Verification items for the finished model (mm, model axes). A direction names the side the tool comes from. Coordinates: 2 decimals unless noted, no trailing zeros. Order: outer loops, then holes, each group sorted by start corner. A loop starts at its lowest first (then second) coordinate and runs counter-clockwise, first axis right, second up. Notation, with made-up numbers: M 59.25,-2.75 L 89.25,-2.75 A34 ccw 89.25,28.25 Z; hole C -27,2.25 d5. An arc over 180 degrees is marked long. Return JSON: item names as keys, results as strings. Group by question number.
Q1. Access from +Z, -Z, +X, -X, +Y, -Y to the whole of each face (thin tool, end or side, straight path). Record for faces 1 (the face through (5.3, 0.2, 0)), 2 (the face through (11.215, 11.199, -3.042)).
Q2. Section check A-A, the plane y = 0. Enter the section's corners in (x, z), then the cut area to 3 significant figures.
Q3. Section check D-D, the plane y = 9. Enter the section's corners in (x, z), then the cut area to 3 significant figures.
Q4. Thickness scan on probe 1 along Z at (x, y) = (-0.75, -8.5); probe 2 along Y at (x, z) = (4, 14.5); probe 3 along Y at (x, z) = (4.5, 7). Record the ranges inside material, lowest first.
Q5. Section check C-C, the plane z = 21.5. Enter the section's corners in (x, y), then the cut area to 3 significant figures.
Q6. Go/stop test with flat-tipped pins: pin 1 Ø6 at (y, z) = (-6, 4.5) entering from +X; pin 2 Ø2 at (x, z) = (3, 15) entering from +Y; pin 3 Ø3 at (y, z) = (6, 10.5) entering from -X; pin 4 Ø11.5 at (x, y) = (-5.5, 3) entering from +Z. Record where each tip stops, or that it passes through.
from build123d import *

# Parameters (mm, degrees)
SKETCH_1_R      = 5
EXTRUDE_1_DEPTH = 25
SKETCH_2_W      = 23
SKETCH_2_H      = 23
EXTRUDE_2_DEPTH = 6
FILLET_1_R      = 1


with BuildPart() as part:
    # 草图1 → 凸台-拉伸1 (new body)
    with BuildSketch(Plane.XY):
        Circle(SKETCH_1_R)
    extrude(amount=EXTRUDE_1_DEPTH)

    # 草图2 → 凸台-拉伸2 (add)
    with BuildSketch(Plane(origin=(0, 0, 0), x_dir=(-1, 0, 0), z_dir=(0, 0, -1))):
        Rectangle(SKETCH_2_W, SKETCH_2_H)
    extrude(amount=EXTRUDE_2_DEPTH)

    # 圆角1
    fillet_1_edges = [part.edges().sort_by_distance(p)[0] for p in [
        (11.5, 11.5, -3),
        (11.5, -11.5, -3),
        (-11.5, -11.5, -3),
        (-11.5, 11.5, -3),
    ]]
    fillet(fillet_1_edges, radius=FILLET_1_R)


solid = part.part
Numbers:
{
 "1": {"face 1": "+Z", "face 2": "+Z, -Z, +X, +Y"},
 "2": {"outline": "M -11.5,-6 L 11.5,-6 L 11.5,0 L 5,0 L 5,25 L -5,25 L -5,0 L -11.5,0 Z", "area": "388 mm2"},
 "3": {"outline": "M -11.5,-6 L 11.5,-6 L 11.5,0 L -11.5,0 Z", "area": "138 mm2"},
 "4": {"probe 1": "z = -6 to 0", "probe 2": "y = -3 to 3", "probe 3": "y = -2.18 to 2.18"},
 "5": {"outline": "C 0,0 d10", "area": "78.5 mm2"},
 "6": {"pin 1": "stops at x = 4", "pin 2": "stops at y = 4.58", "pin 3": "stops at x = -2.18", "pin 4": "stops at z = 25"}
}
